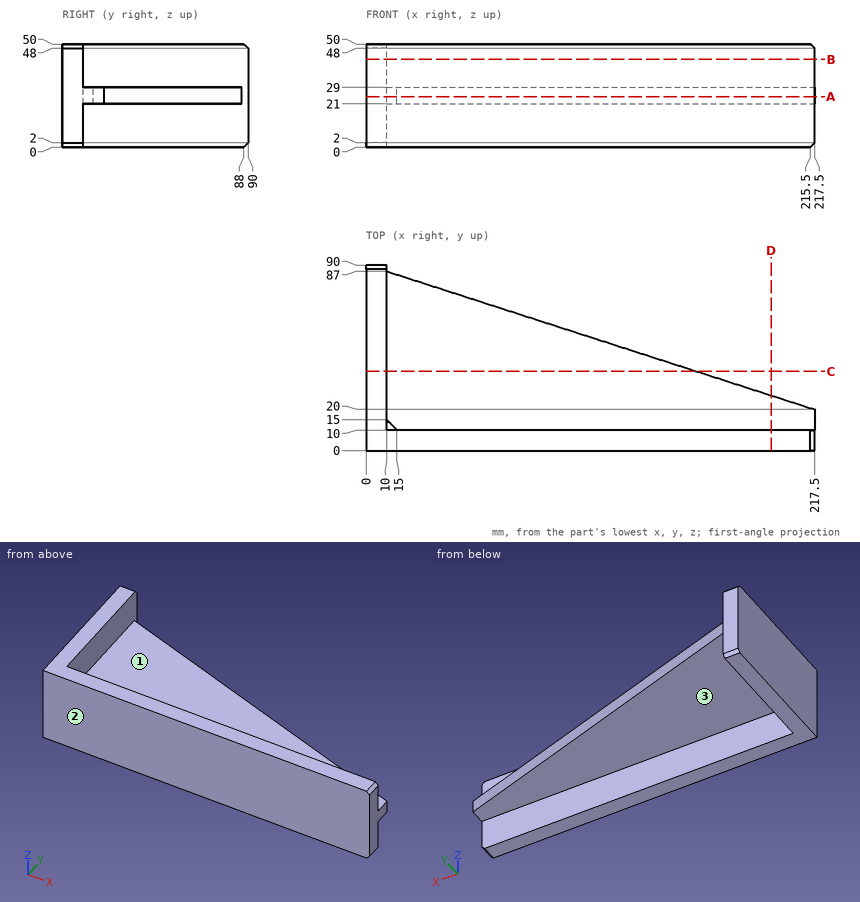
Here's the drawing with two shaded views (mm, measured from the low corner). I have some questions. A direction names the side the tool comes from. Coordinates: 2 decimals unless noted, no trailing zeros. Write each loop counter-clockwise with the first axis right and the second up, starting at its lowest first coordinate (ties: lowest second). Pieces come first, ordered by that corner, then holes. Notation, with made-up numbers: (53.5, 52) - (71.5, 52) arc R28 ccw to (71.5, 76) - close; hole circle Ø7 at (-20, 42). An arc over 180 degrees is marked (long way). Return JSON: item names as keys, results as strings.
Q1. I'm going to push flat-ended pins straight in: pin 1 Ø3 at (y, z) = (37.5, 34) entering from -X; pin 2 Ø4 at (x, y) = (170.5, 33.5) entering from -Z; pin 3 Ø5 at (x, z) = (112, 12.5) entering from +Y; pin 4 Ø2 at (y, z) = (77, 6) entering from +X. Where does each tip first touch, or does it pass through?
Computed values:
{"pin 1": "stops at x = 0", "pin 2": "stops at z = 21", "pin 3": "stops at y = 10", "pin 4": "stops at x = 10"}
Q2. Please list where these lines run through material, in increasing order: L1, parallel to Y at x = 42, z = 43.5; L2, parallel to Z at x = 143.5, y = 23. Write a range as from..to.
Computed values:
{"L1": "y = 0..10", "L2": "z = 21..29"}
Q3. If we section it at A-A (z = 24.5): Please give me the cut outline in (x, y), then the cut area to 3 significant figures.
Computed values:
{"outline": "(0, 0) - (217.5, 0) - (217.5, 20) - (10, 87) - (10, 90) - (0, 90) - close; hole (10, 10) - (15, 10) - (10, 15) - close", "area": "12,000 mm2"}
Q4. If we section it at C-C (y = 38.5): Please give me the cut outline in (x, z).
Computed values:
{"outline": "(0, 0) - (10, 0) - (10, 21) - (160.21, 21) - (160.21, 29) - (10, 29) - (10, 50) - (0, 50) - close"}
Q5. If we section it at D-D (x = 196.5): Please give me the cut outline in (y, z).
Computed values:
{"outline": "(0, 0) - (10, 0) - (10, 21) - (26.78, 21) - (26.78, 29) - (10, 29) - (10, 50) - (0, 50) - close"}
Q6. If we section it at B-B (z = 42.5): Please give me the cut outline in (x, y).
Computed values:
{"outline": "(0, 0) - (217.5, 0) - (217.5, 10) - (10, 10) - (10, 90) - (0, 90) - close"}
Q7. On a 3-axis mill with a long thin cutter (end or side, diameter ignored), from which of +Z, -Z, +X, -X, +Y, -Y can I reach the whole of each face in a straight line? I mean the marked faces 1, 2 and 3. Say none if no direction works.
Computed values:
{"face 1": "+Z, +X, +Y", "face 2": "+Z, -Z, +X, -X, -Y", "face 3": "-Z, +X, +Y"}
